The model under review builds one solid part; all positions refer to its coordinate system, in mm. Round coordinates to 2 decimals unless told otherwise and drop trailing zeros. Write each loop counter-clockwise with the first axis right and the second up, starting at its lowest first coordinate (ties: lowest second). Pieces come first, ordered by that corner, then holes. Notation, with made-up numbers: (-25.5, 31) -> (18.5, 31) arc R11 cw to (18.5, 46) -> close; hole circle Ø10 at (81, 55.25). An arc over 180 degrees is marked (long way). Return JSON: item names as keys, results as strings. Group by question number.
1. For line 1 along Y through (x, z) = (-48, 4.55); line 2 along X through (y, z) = (-63, 1.6); line 3 along Y through (x, z) = (73, 3.5), list the stretches that pass through material, from the lowest coordinate up. Write a range as from..to.
2. Take a section at B-B, the plane z = 3.25. Write out the cut boundary in (x, y), then the cut area to 3 significant figures.
3. Take a section at C-C, the plane y = 55. Write out the cut boundary in (x, z).
4. Mouldability with a two-part tool opening along X and no side actions: class faces 1 (the cylindrical face through (68.84, -64.22, 2.96)), 2 (the flat face through (-1, 1, 6)), 3 (the flat face through (-103, -1, 3)), 4 (the flat face through (103, -28, 3)) as pulls with the +X half, pulls with the -X half, needs draft (parallel to the pull), parting line crosses it, or undercut.
5. Clearance check with a flat-ended pin moving along its axis: P1, Ø5.5, axis at x = 46, y = 15.5, coming from the -Z side. State where the tip first meets the part, or that it passes through.
6. Take a section at A-A, the plane x = -88. Write out the cut boundary in (y, z), then the cut area to 3 significant figures.
7. Take a section at D-D, the plane x = 73. Write out the cut boundary in (y, z).
from build123d import *

# Parameters (mm, degrees)
SKETCH_1_W          = 206
SKETCH_1_H          = 145
EXTRUDE_1_DEPTH     = 6
SKETCH_3_R          = 4.5
CUT_EXTRUDE_2_DEPTH = 127.100158604
SKETCH_4_R          = 4.5
CUT_EXTRUDE_3_DEPTH = 127.100158604
FILLET_4_R          = 57
SKETCH_10_R         = 4.5
CUT_EXTRUDE_6_DEPTH = 10
FILLET_6_R          = 3


with BuildPart() as part:
    # 草图1 → 凸台-拉伸1 (new body)
    with BuildSketch(Plane.XY):
        Rectangle(SKETCH_1_W, SKETCH_1_H)
    extrude(amount=EXTRUDE_1_DEPTH)

    # 草图3 → 切除-拉伸2 (cut, through all)
    with BuildSketch(Plane.XY.offset(6)):
        with Locations((-88, 55)):
            Circle(SKETCH_3_R)
        with Locations((-48, 55)):
            Circle(SKETCH_3_R)
        with Locations((-88, -62.5)):
            Circle(SKETCH_3_R)
        with Locations((-48, -62.5)):
            Circle(SKETCH_3_R)
    extrude(amount=-CUT_EXTRUDE_2_DEPTH, mode=Mode.SUBTRACT)

    # 草图4 → 切除-拉伸3 (cut, through all)
    with BuildSketch(Plane.XY.offset(6)):
        with Locations((46, 15.5)):
            Circle(SKETCH_4_R)
    extrude(amount=-CUT_EXTRUDE_3_DEPTH, mode=Mode.SUBTRACT)

    # 圆角4
    fillet_4_edges = [part.edges().sort_by_distance(p)[0] for p in [
        (103, 72.5, 3),
    ]]
    fillet(fillet_4_edges, radius=FILLET_4_R)

    # 草图10 → 切除-拉伸6 (cut)
    with BuildSketch(Plane(origin=(0, 0, 0), x_dir=(-1, 0, 0), z_dir=(0, 0, -1))):
        with Locations((-73, -62.5)):
            Circle(SKETCH_10_R)
    extrude(amount=-CUT_EXTRUDE_6_DEPTH, mode=Mode.SUBTRACT)

    # 圆角6
    fillet_6_edges = [part.edges().sort_by_distance(p)[0] for p in [
        (103, -72.5, 3),
    ]]
    fillet(fillet_6_edges, radius=FILLET_6_R)


solid = part.part
Output:
{
 "1": {"line 1": "y = -72.5..-67, -58..50.5, 59.5..72.5", "line 2": "x = -103..-92.47, -83.53..-52.47, -43.53..68.53, 77.47..103", "line 3": "y = -72.5..-67, -58..65.7"},
 "2": {"outline": "(-103, -72.5) -> (100, -72.5) arc R3 ccw to (103, -69.5) -> (103, 15.5) arc R57 ccw to (46, 72.5) -> (-103, 72.5) -> close; hole circle Ø9 at (-88, -62.5); hole circle Ø9 at (-88, 55); hole circle Ø9 at (-48, -62.5); hole circle Ø9 at (-48, 55); hole circle Ø9 at (46, 15.5); hole circle Ø9 at (73, -62.5)", "area": "28,800 mm^2"},
 "3": {"outline": "(-103, 0) -> (-92.5, 0) -> (-92.5, 6) -> (-103, 6) -> close; (-83.5, 0) -> (-52.5, 0) -> (-52.5, 6) -> (-83.5, 6) -> close; (-43.5, 0) -> (87.09, 0) -> (87.09, 6) -> (-43.5, 6) -> close"},
 "4": {"face 1": "undercut", "face 2": "needs draft", "face 3": "pulls with the -X half", "face 4": "pulls with the +X half"},
 "5": {"P1": "passes through"},
 "6": {"outline": "(-72.5, 0) -> (-67, 0) -> (-67, 6) -> (-72.5, 6) -> close; (-58, 0) -> (50.5, 0) -> (50.5, 6) -> (-58, 6) -> close; (59.5, 0) -> (72.5, 0) -> (72.5, 6) -> (59.5, 6) -> close", "area": "762 mm^2"},
 "7": {"outline": "(-72.5, 0) -> (-67, 0) -> (-67, 6) -> (-72.5, 6) -> close; (-58, 0) -> (65.7, 0) -> (65.7, 6) -> (-58, 6) -> close"}
}
